```python
from build123d import *

# Parameters (mm, degrees)
SKETCH1_W                                           = 200
SKETCH1_H                                           = 183
BOSS_EXTRUDE1_DEPTH                                 = 15
M8_TAPPED_HOLE1_D                                   = 6.8
SKETCH11_W                                          = 200
SKETCH11_H                                          = 15
BOSS_EXTRUDE3_DEPTH                                 = 15
CBORE_FOR_M6_HEX_SOCKET_HEAD_CAP_SCREW1_D           = 6.6
CBORE_FOR_M6_HEX_SOCKET_HEAD_CAP_SCREW1_CBORE_D     = 11
CBORE_FOR_M6_HEX_SOCKET_HEAD_CAP_SCREW1_CBORE_DEPTH = 6
CBORE_FOR_M8_HEX_SOCKET_HEAD_CAP_SCREW1_D           = 9
CBORE_FOR_M8_HEX_SOCKET_HEAD_CAP_SCREW1_CBORE_D     = 15
CBORE_FOR_M8_HEX_SOCKET_HEAD_CAP_SCREW1_CBORE_DEPTH = 8.6
SKETCH9_W                                           = 200
SKETCH9_H                                           = 15
BOSS_EXTRUDE2_DEPTH                                 = 5
SKETCH10_R                                          = 4
CUT_EXTRUDE2_DEPTH                                  = 147.857924539
CHAMFER1_SIZE                                       = 5
SKETCH12_R                                          = 55
CUT_EXTRUDE3_DEPTH                                  = 147.857924539


with BuildPart() as part:
    # Sketch1 → Boss-Extrude1 (new body)
    with BuildSketch(Plane(origin=(0, 0, 0), x_dir=(1, 0, 0), z_dir=(0, 1, 0))):
        Rectangle(SKETCH1_W, SKETCH1_H)
    extrude(amount=BOSS_EXTRUDE1_DEPTH)

    # M8 Tapped Hole1 (through all)
    with Locations(Plane(origin=(0, 15, 0), x_dir=(-1, 0, 0), z_dir=(0, 1, 0))):
        with Locations((35.461940777, -62.461940777), (-56.461940777, -62.461940777), (35.461940777, 29.461940777), (-56.461940777, 29.461940777)):
            Hole(M8_TAPPED_HOLE1_D / 2)

    # Sketch11 → Boss-Extrude3 (add)
    with BuildSketch(Plane(origin=(0, 0, -91.5), x_dir=(-1, 0, 0), z_dir=(0, 0, -1))):
        with Locations((0, 7.5)):
            Rectangle(SKETCH11_W, SKETCH11_H)
    extrude(amount=BOSS_EXTRUDE3_DEPTH)

    # CBORE for M6 Hex Socket Head Cap Screw1 (through all)
    with Locations(Plane(origin=(0, 15, 0), x_dir=(-1, 0, 0), z_dir=(0, 1, 0))):
        with Locations((-70, -99), (10, -99)):
            CounterBoreHole(CBORE_FOR_M6_HEX_SOCKET_HEAD_CAP_SCREW1_D / 2, CBORE_FOR_M6_HEX_SOCKET_HEAD_CAP_SCREW1_CBORE_D / 2, CBORE_FOR_M6_HEX_SOCKET_HEAD_CAP_SCREW1_CBORE_DEPTH)

    # CBORE for M8 Hex Socket Head Cap Screw1 (through all)
    with Locations(Plane(origin=(0, 15, 0), x_dir=(-1, 0, 0), z_dir=(0, 1, 0))):
        with Locations((-85, 35.5), (80, 35.5)):
            CounterBoreHole(CBORE_FOR_M8_HEX_SOCKET_HEAD_CAP_SCREW1_D / 2, CBORE_FOR_M8_HEX_SOCKET_HEAD_CAP_SCREW1_CBORE_D / 2, CBORE_FOR_M8_HEX_SOCKET_HEAD_CAP_SCREW1_CBORE_DEPTH)

    # Sketch9 → Boss-Extrude2 (add)
    with BuildSketch(Plane.XY.offset(91.5)):
        with Locations((0, 7.5)):
            Rectangle(SKETCH9_W, SKETCH9_H)
    extrude(amount=BOSS_EXTRUDE2_DEPTH)

    # Sketch10 → Cut-Extrude2 (cut, through all)
    with BuildSketch(Plane(origin=(0, 15, 0), x_dir=(1, 0, 0), z_dir=(0, 1, 0))):
        with Locations(Location((-80, -85.5, 0), (0, 0, 270))):
            Circle(SKETCH10_R)
        with Locations(Location((80, -85.5, 0), (0, 0, 270))):
            Circle(SKETCH10_R)
    extrude(amount=-CUT_EXTRUDE2_DEPTH, mode=Mode.SUBTRACT)

    # Chamfer1
    chamfer1_edges = [part.edges().sort_by_distance(p)[0] for p in [
        (-100, 7.5, 96.5),
        (100, 7.5, 96.5),
    ]]
    chamfer(chamfer1_edges, length=CHAMFER1_SIZE)

    # Sketch12 → Cut-Extrude3 (cut, through all)
    with BuildSketch(Plane(origin=(0, 15, 0), x_dir=(1, 0, 0), z_dir=(0, 1, 0))):
        with Locations(Location((10.5, 16.5, 0), (0, 0, 270))):
            Circle(SKETCH12_R)
    extrude(amount=-CUT_EXTRUDE3_DEPTH, mode=Mode.SUBTRACT)


solid = part.part
```
The model under review builds one solid part; all positions refer to its coordinate system, in mm. A direction names the side the tool comes from. Round coordinates to 2 decimals unless told otherwise and drop trailing zeros. Order: outer loops, then holes, each group sorted by start corner. A loop starts at its lowest first (then second) coordinate and runs counter-clockwise, first axis right, second up.
(1) For P1, Ø8.5, axis at x = -10, z = -99, coming from the +Y side; P2, Ø11.5, axis at x = -80, z = 35.5, coming from the +Y side, all flat-tipped, find the tip position at first contact; note any pin that passes through.
Working result:
P1: stops at y = 9
P2: stops at y = 6.4
(2) Take a section at D-D, the plane x = 10.5. State the section outline as (y, z) points, plus the area to 4 significant figures.
Working result:
outline: (0, -106.5) - (15, -106.5) - (15, -71.5) - (0, -71.5) - close; (0, 38.5) - (15, 38.5) - (15, 96.5) - (0, 96.5) - close
area: 1,395 mm2
(3) Wall thickness on L1, parallel to X at y = 12, z = -61; L2, parallel to Z at x = -79, y = 13.5; L3, parallel to Z at x = 70, y = 11: over which ranges is each line inside the solid? List them lowest first.
Working result:
L1: x = -100 to -38.53, -32.39 to -21.82, 42.82 to 53.39, 59.53 to 100
L2: z = -106.5 to 28.07, 42.93 to 81.63, 89.37 to 96.5
L3: z = -106.5 to -104.5, -93.5 to 96.5
(4) Take a section at B-B, the plane z = 85.5. State the section outline as (x, y) points.
Working result:
outline: (-100, 0) - (-84, 0) - (-84, 15) - (-100, 15) - close; (-76, 0) - (76, 0) - (76, 15) - (-76, 15) - close; (84, 0) - (100, 0) - (100, 15) - (84, 15) - close
(5) Take a section at A-A, the plane x = -80. State the section outline as (y, z) points.
Working result:
outline: (0, -106.5) - (15, -106.5) - (15, 28) - (6.4, 28) - (6.4, 31) - (0, 31) - close; (0, 40) - (6.4, 40) - (6.4, 43) - (15, 43) - (15, 81.5) - (0, 81.5) - close; (0, 89.5) - (15, 89.5) - (15, 96.5) - (0, 96.5) - close
(6) Tool access review of faces 1 (the face through (81.4, 3.2, 32.8)), 2 (the face through (85.1, 6.4, 30.6)): name each direction out of +Z, -Z, +X, -X, +Y, -Y from which nothing blocks a thin tool from reaching the whole face with its end or side.
Working result:
face 1: +Y, -Y
face 2: +Y
(7) Mouldability with a two-part tool opening along Z and no side actions: class faces 3 (the face through (1, 8, -106.5)), 4 (the face through (97.5, 7.4, 94)), 5 (the face through (-85, 6.4, 36)) as released by +Z, released by -Z, zero draft, split by the parting line, or undercut.
Working result:
face 3: released by -Z
face 4: released by +Z
face 5: undercut
(8) Take a section at C-C, the plane z = -16.5. State the section outline as (x, y) points.
Working result:
outline: (-100, 0) - (-44.5, 0) - (-44.5, 15) - (-100, 15) - close; (65.5, 0) - (100, 0) - (100, 15) - (65.5, 15) - close
